Source: CAD feature listing. Evaluate the final solid. Frame: model axes, mm. Face numbers are marked on the shaded views. A direction names the side the tool comes from. Round coordinates to 2 decimals unless told otherwise and drop trailing zeros. Write each loop counter-clockwise with the first axis right and the second up, starting at its lowest first coordinate (ties: lowest second). Pieces come first, ordered by that corner, then holes. Notation, with made-up numbers: (33, 28.5) -> (70, 28.5) arc R36 cw to (70, 66.5) -> close; hole circle Ø6 at (82, 16.25). An arc over 180 degrees is marked (long way). Put each result on its own line as item: value.
```python
from build123d import *

# Parameters (mm, degrees)
SKETCH_1_W                  = 50
SKETCH_1_H                  = 45
EXTRUDE_1_DEPTH             = 10
SKETCH_2_W                  = 49.938204031
SKETCH_2_H                  = 20
EXTRUDE_2_DEPTH             = 35
HOLE_WIZARD_20_5_20_5_1_D   = 20.5
SKETCH_6_W                  = 3.4
SKETCH_6_H                  = 10
HOLE_WIZARD_M8_1_AT_2_COUNT = 2
HOLE_WIZARD_M8_1_AT_2_PITCH = 25
HOLE_WIZARD_M8_1_AT_3_COUNT = 2
HOLE_WIZARD_M8_1_AT_3_PITCH = 30
HOLE_WIZARD_M8_1_AT_4_COUNT = 2
HOLE_WIZARD_M8_1_AT_4_PITCH = 39.05124838
CHAMFER_1_SIZE              = 10
CHAMFER_2_SIZE              = 5


with BuildPart() as part:
    # 草图1 → 凸台-拉伸1 (new body)
    with BuildSketch(Plane(origin=(0, 0, 0), x_dir=(0, 0, -1), z_dir=(1, 0, 0))):
        Rectangle(SKETCH_1_W, SKETCH_1_H)
    extrude(amount=EXTRUDE_1_DEPTH)

    # 草图2 → 凸台-拉伸2 (add)
    with BuildSketch(Plane(origin=(10, 0, 0), x_dir=(0, 0, -1), z_dir=(1, 0, 0))):
        with Locations((0.030897984, -12.5)):
            Rectangle(SKETCH_2_W, SKETCH_2_H)
    extrude(amount=EXTRUDE_2_DEPTH)

    # Ø20.5 (20.5) 直径孔1 (through all)
    with Locations(Plane(origin=(0, -22.5, 0), x_dir=(-1, 0, 0), z_dir=(0, -1, 0))):
        with Locations((-25, 0)):
            Hole(HOLE_WIZARD_20_5_20_5_1_D / 2)

    # 草图6 → M8 螺纹孔1 (revolve, cut)
    with BuildSketch(Plane(origin=(10, 16.5, 12.5), x_dir=(0, 0, -1), z_dir=(0, 1, 0))):
        with Locations((1.7, 5)):
            Rectangle(SKETCH_6_W, SKETCH_6_H)
    hole_wizard_m8_1 = revolve(axis=Axis((16.35, 16.5, 12.5), (-1, 0, 0)), mode=Mode.SUBTRACT)

    # M8 螺纹孔1 at 2: M8 螺纹孔1 ×2
    with Locations(*[(0, 0, -i * HOLE_WIZARD_M8_1_AT_2_PITCH) for i in range(1, HOLE_WIZARD_M8_1_AT_2_COUNT)]):
        add(hole_wizard_m8_1, mode=Mode.SUBTRACT)

    # M8 螺纹孔1 at 3: M8 螺纹孔1 ×2
    with Locations(*[(0, -i * HOLE_WIZARD_M8_1_AT_3_PITCH, 0) for i in range(1, HOLE_WIZARD_M8_1_AT_3_COUNT)]):
        add(hole_wizard_m8_1, mode=Mode.SUBTRACT)

    # M8 螺纹孔1 at 4: M8 螺纹孔1 ×2
    with Locations(*[Vector(0, -0.7682212795973759, -0.64018439966448) * (i * HOLE_WIZARD_M8_1_AT_4_PITCH) for i in range(1, HOLE_WIZARD_M8_1_AT_4_COUNT)]):
        add(hole_wizard_m8_1, mode=Mode.SUBTRACT)

    # 倒角1
    chamfer_1_edges = [part.edges().sort_by_distance(p)[0] for p in [
        (45, -12.5, -25),
        (45, -12.5, 24.938204031),
    ]]
    chamfer(chamfer_1_edges, length=CHAMFER_1_SIZE)

    # 倒角2
    chamfer_2_edges = [part.edges().sort_by_distance(p)[0] for p in [
        (5, 22.5, 25),
        (5, 22.5, -25),
    ]]
    chamfer(chamfer_2_edges, length=CHAMFER_2_SIZE)


solid = part.part
```
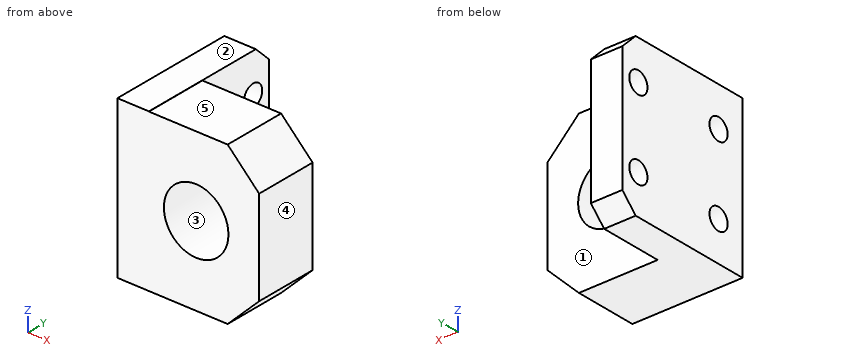
Q1. Cut plane C-C on x = 25. Output: boundary loops of the cut face in (y, z).
Ans:
outline: (-22.5, -25) -> (-2.5, -25) -> (-2.5, -10.25) -> (-22.5, -10.25) -> close; (-22.5, 10.25) -> (-2.5, 10.25) -> (-2.5, 24.94) -> (-22.5, 24.94) -> close
Q2. Reachability of the marked faces 1 and 2 from +Z, -Z, +X, -X, +Y, -Y: full face, straight path, thin tool, end or side. Return the list, or none.
Ans:
face 1: +Z, -Z, +X, +Y
face 2: +Z, +X, -X, +Y, -Y
Q3. Cut plane B-B on z = 12.5. Output: boundary loops of the cut face in (x, y).
Ans:
outline: (0, -22.5) -> (45, -22.5) -> (45, -2.5) -> (10, -2.5) -> (10, 13.1) -> (0, 13.1) -> (0, -10.1) -> (10, -10.1) -> (10, -16.9) -> (0, -16.9) -> close; (0, 19.9) -> (10, 19.9) -> (10, 22.5) -> (0, 22.5) -> close
Q4. Pin query (flat end, axial travel): pin 1 (10 mm diameter, centred on x = 17, y = -16, fed in from +Z); pin 2 (1 mm diameter, centred on x = 32.5, z = -18.5, fed in from +Y); pin 3 (3 mm diameter, centred on x = 26, z = 8.5, fed in from +Y); pin 4 (5.5 mm diameter, centred on y = -13.5, z = 12.5, fed in from -X). Return the tip coordinate at first contact, or that it passes through.
Ans:
pin 1: stops at z = 24.94
pin 2: stops at y = -2.5
pin 3: passes through
pin 4: stops at x = 10
Q5. Cut plane A-A on y = 16.5. Output: boundary loops of the cut face in (x, z), and give its area (3 significant figures).
Ans:
outline: (0, -25) -> (10, -25) -> (10, -15.9) -> (0, -15.9) -> close; (0, -9.1) -> (10, -9.1) -> (10, 9.1) -> (0, 9.1) -> close; (0, 15.9) -> (10, 15.9) -> (10, 25) -> (0, 25) -> close
area: 364 mm^2
Q6. Cut plane D-D on y = -13.5. Output: boundary loops of the cut face in (x, z).
Ans:
outline: (0, -25) -> (35, -25) -> (45, -15) -> (45, 14.94) -> (35, 24.94) -> (10, 24.94) -> (10, 25) -> (0, 25) -> (0, 15.9) -> (10, 15.9) -> (10, 9.1) -> (0, 9.1) -> (0, -9.1) -> (10, -9.1) -> (10, -15.9) -> (0, -15.9) -> close; hole circle Ø20.5 at (25, 0)
Q7. Material intervals for line 1 (Y direction, x = 3, z = -12.5); line 2 (Z direction, x = 6.5, y = -13.5); line 3 (X direction, y = -18.5, z = 0.5), sorted ascending. Write a range as [from, to].
Ans:
line 1: y = [-22.5, -16.9], [-10.1, 13.1], [19.9, 22.5]
line 2: z = [-25, -15.9], [-9.1, 9.1], [15.9, 25]
line 3: x = [0, 14.76], [35.24, 45]
Q8. Draft query along Z for the marked faces 3, 4 and 5. Return one class per face: +Z half, -Z half, draft (parallel to the pull), parting line (faces both ways), or undercut.
Ans:
face 3: undercut
face 4: draft
face 5: +Z half
